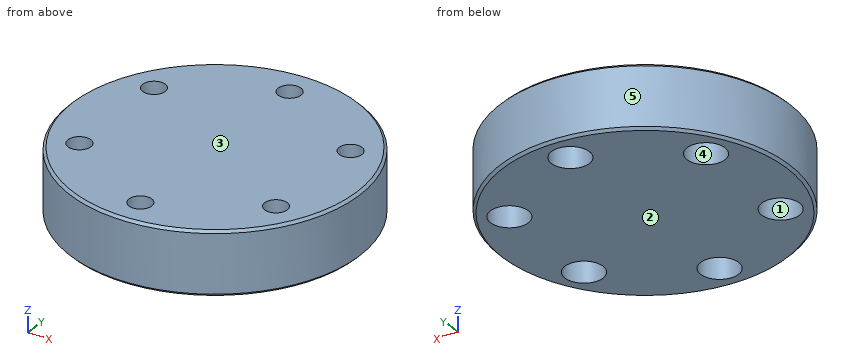
```python
from build123d import *

# Parameters (mm, degrees)
SKETCH1_R                                           = 57
BOSS_EXTRUDE1_DEPTH                                 = 25
CHAMFER3_SIZE                                       = 1
HOLE_SIZE_PER_SOCKET_HEAD_CAP_SCREW_TYP_D           = 9
HOLE_SIZE_PER_SOCKET_HEAD_CAP_SCREW_TYP_CBORE_D     = 15
HOLE_SIZE_PER_SOCKET_HEAD_CAP_SCREW_TYP_CBORE_DEPTH = 12
CIRPATTERN1_COUNT                                   = 6


with BuildPart() as part:
    # Sketch1 → Boss-Extrude1 (new body)
    with BuildSketch(Plane.XY):
        Circle(SKETCH1_R)
    extrude(amount=BOSS_EXTRUDE1_DEPTH)

    # Chamfer3
    chamfer3_edges = [part.edges().sort_by_distance(p)[0] for p in [
        (-57, 0, 0),
        (-57, 0, 25),
    ]]
    chamfer(chamfer3_edges, length=CHAMFER3_SIZE)

    # Hole size (per socket head cap screw type)1 (through all)
    with Locations(Plane(origin=(0, 0, 0), x_dir=(-1, 0, 0), z_dir=(0, 0, -1))):
        with Locations((0, 45)):
            hole_size_per_socket_head_cap_screw_typ = CounterBoreHole(HOLE_SIZE_PER_SOCKET_HEAD_CAP_SCREW_TYP_D / 2, HOLE_SIZE_PER_SOCKET_HEAD_CAP_SCREW_TYP_CBORE_D / 2, HOLE_SIZE_PER_SOCKET_HEAD_CAP_SCREW_TYP_CBORE_DEPTH)

    # CirPattern1: Hole size (per socket head cap screw type)1 ×6 about axis
    cirpattern1_axis = Axis((0, 0, 0), (0, 0, 1))
    for i in range(1, CIRPATTERN1_COUNT):
        add(hole_size_per_socket_head_cap_screw_typ.rotate(cirpattern1_axis, i * 360 / CIRPATTERN1_COUNT), mode=Mode.SUBTRACT)


solid = part.part
```
Geometry check sheet. Reference: the model listing, model coordinates, mm. Face numbers are marked on the shaded views. A direction names the side the tool comes from. Give positions to 0.01 mm unless a question says otherwise; leave off trailing zeros. Order: outer loops, then holes, each group sorted by start corner. A loop starts at its lowest first (then second) coordinate and runs counter-clockwise, first axis right, second up. Notation, with made-up numbers: (-15, 35) - (-7, 35) arc R34 cw to (-7, 71) - close; hole circle Ø5 at (82, -9). An arc over 180 degrees is marked (long way). Answer in a Markdown table with one row per item. Add a question column.
Q1. Cross-section at D-D, the plane z = 17.75. Enter the section's corners in (x, y), then the cut area to 3 significant figures.
Q2. Cross-section at B-B, the plane z = 10.5. Enter the section's corners in (x, y).
Q3. Tool access check on the marked faces 1 and 2. Record the directions out of +Z, -Z, +X, -X, +Y, -Y that give a thin tool (end or side, any length) a straight path to the whole face; none if there is none.
Q4. Material ranges on probe 1 along Y at (x, z) = (0, 6.75); probe 2 along Y at (x, z) = (0, 19.25); probe 3 along X at (y, z) = (-19.5, 14.5), recorded low to high. Write a range as from..to.
Q5. Gauge pin test, flat ends, axial feed: pin 1 (3 mm diameter, centred on x = -44.5, y = -40.5, fed in from +Z) (3 decimals); pin 2 (6 mm diameter, centred on x = 36, y = -24, fed in from -Z); pin 3 (1 mm diameter, centred on y = -10, z = 18, fed in from -X); pin 4 (3 mm diameter, centred on x = 21, z = 10.5, fed in from -Y). Record the tip position at first contact, or that the pin passes through.
Q6. Cross-section at A-A, the plane x = 0. Enter the section's corners in (y, z), then the cut area to 3 significant figures.
Q7. Mould release check, pull along X, two halves, no side actions. Record for the marked faces 3, 4 and 5: pulls with the +X half, pulls with the -X half, needs draft (parallel to the pull), parting line crosses it, or undercut.
Q8. Cross-section at C-C, the plane y = -22.5. Count the separate pieces of the cut face and the enclosed holes in it, then the cut area to 3 significant figures.
Check values:
| question | item | result |
|---|---|---|
| 1 | outline | circle Ø114 at (0, 0); hole circle Ø9 at (-38.97, -22.5); hole circle Ø9 at (-38.97, 22.5); hole circle Ø9 at (0, -45); hole circle Ø9 at (0, 45); hole circle Ø9 at (38.97, -22.5); hole circle Ø9 at (38.97, 22.5) |
| 1 | area | 9,830 mm^2 |
| 2 | outline | circle Ø114 at (0, 0); hole circle Ø15 at (-38.97, -22.5); hole circle Ø15 at (-38.97, 22.5); hole circle Ø15 at (0, -45); hole circle Ø15 at (0, 45); hole circle Ø15 at (38.97, -22.5); hole circle Ø15 at (38.97, 22.5) |
| 3 | face 1 | -Z |
| 3 | face 2 | -Z, +X, -X, +Y, -Y |
| 4 | probe 1 | y = -57..-52.5, -37.5..37.5, 52.5..57 |
| 4 | probe 2 | y = -57..-49.5, -40.5..40.5, 49.5..57 |
| 4 | probe 3 | x = -53.56..-42.33, -35.62..35.62, 42.33..53.56 |
| 5 | pin 1 | passes through |
| 5 | pin 2 | stops at z = 12 |
| 5 | pin 3 | stops at x = -56.2 |
| 5 | pin 4 | stops at y = -53.56 |
| 6 | outline | (-57, 1) - (-56, 0) - (-52.5, 0) - (-52.5, 12) - (-49.5, 12) - (-49.5, 25) - (-56, 25) - (-57, 24) - close; (-40.5, 12) - (-37.5, 12) - (-37.5, 0) - (37.5, 0) - (37.5, 12) - (40.5, 12) - (40.5, 25) - (-40.5, 25) - close; (49.5, 12) - (52.5, 12) - (52.5, 0) - (56, 0) - (57, 1) - (57, 24) - (56, 25) - (49.5, 25) - close |
| 6 | area | 2,250 mm^2 |
| 7 | face 3 | needs draft |
| 7 | face 4 | undercut |
| 7 | face 5 | parting line crosses it |
| 8 | separate pieces | 3 |
| 8 | enclosed holes | 0 |
| 8 | area | 2,020 mm^2 |
